Geometry: final body of the model. Coordinates: model frame, mm. Face numbers are marked on the shaded views. A direction names the side the tool comes from. Give positions to 0.01 mm unless a question says otherwise; leave off trailing zeros. Order: outer loops, then holes, each group sorted by start corner. A loop starts at its lowest first (then second) coordinate and runs counter-clockwise, first axis right, second up. Notation, with made-up numbers: (9, -37) - (44, -37) arc R13 cw to (44, -28) - close; hole circle Ø6 at (-29.5, 63.5). An arc over 180 degrees is marked (long way). Put each result on its own line as item: value. Start each with the question number.
1. Section D-D on y = 75. Return the cut outline in (x, z).
2. Mould query, pull axis Y, two halves, no side actions, for the marked faces 5, 6 and 7. Classes: pulls with the +Y half, pulls with the -Y half, needs draft (parallel to the pull), parting line crosses it, or undercut.
3. First-contact query: P1, Ø1.5, axis at x = -31, y = -5.5, coming from the -Z side; P2, Ø12, axis at y = 60, z = 4, coming from the -X side; P3, Ø7, axis at x = -39.5, z = -9.5, coming from the +Y side. Flat tips, straight axial feed; report the tip coordinate or a pass-through.
4. Section A-A on z = 0. Return the cut outline in (x, y), plus the area to 3 significant figures.
5. Ray query, line 1 along Y through (x, z) = (17, 0); line 2 along Y through (x, z) = (17, 20); line 3 along Z through (x, y) = (-16, -7.5). Return the intervals inside material, ascending. Write a range as from..to.
6. Set-up query: the marked faces 1, 2, 3 and 4. Return all of +Z, -Z, +X, -X, +Y, -Y with unobstructed straight access to the full face (end or side cutting, diameter ignored); none if empty.
7. Section C-C on x = 0. Return the cut outline in (y, z).
8. Section B-B on x = -21.5. Return the cut outline in (y, z), plus the area to 3 significant figures.
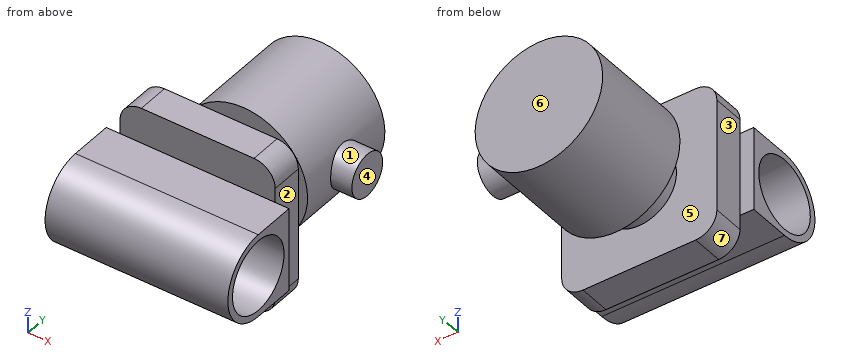
from build123d import *

# Parameters (mm, degrees)
SKETCH_1_R           = 19.75
SKETCH_1_R_2         = 16.75
EXTRUDE_1_DEPTH      = 43
EXTRUDE_1_2_DEPTH    = 15
SKETCH_4_R           = 17.5
EXTRUDE_2_DEPTH      = 15
SKETCH_5_R           = 30
EXTRUDE_3_DEPTH      = 50.25
EXTRUDE_START        = -86
EXTRUDE_4_DEPTH      = 86
EXTRUDE_5_REACH      = 137.171
EXTRUDE_5_END_RADIUS = 30
SKETCH_7_R           = 10


with BuildPart() as part:
    # Sketch 1 → Extrude 1 (new, symmetric)
    with BuildSketch(Plane(origin=(0, 0, 0), x_dir=(0, 0, -1), z_dir=(1, 0, 0))):
        Circle(SKETCH_1_R)
        Circle(SKETCH_1_R_2, mode=Mode.SUBTRACT)
    extrude(amount=EXTRUDE_1_DEPTH, both=True)



with BuildPart() as body_2:
    # Sketch 3 → Extrude 1 2 (new body)
    with BuildSketch(Plane(origin=(0, 20, 0), x_dir=(1, 0, 0), z_dir=(0, 1, 0))):
        with BuildLine():
            Line((-26.5, 36.5), (26.5, 36.5))
            ThreePointArc((26.5, 36.5), (33.571067812, 33.571067812), (36.5, 26.5))
            Line((36.5, 26.5), (36.5, -26.5))
            ThreePointArc((36.5, -26.5), (33.571067812, -33.571067812), (26.5, -36.5))
            Line((26.5, -36.5), (-26.5, -36.5))
            ThreePointArc((-26.5, -36.5), (-33.571067812, -33.571067812), (-36.5, -26.5))
            Line((-36.5, -26.5), (-36.5, 26.5))
            ThreePointArc((-36.5, 26.5), (-33.571067812, 33.571067812), (-26.5, 36.5))
        make_face()
    extrude(amount=EXTRUDE_1_2_DEPTH)

    # Sketch 4 → Extrude 2 (add)
    with BuildSketch(Plane(origin=(0, 35, 0), x_dir=(1, 0, 0), z_dir=(0, 1, 0))):
        with Locations(Location((0, 0, 0), (0, 0, 90))):
            Circle(SKETCH_4_R)
    extrude(amount=EXTRUDE_2_DEPTH)

    # Sketch 5 → Extrude 3 (add)
    with BuildSketch(Plane(origin=(0, 50, 0), x_dir=(1, 0, 0), z_dir=(0, 1, 0))):
        with Locations(Location((0, 0, 0), (0, 0, 270))):
            Circle(SKETCH_5_R)
    extrude(amount=EXTRUDE_3_DEPTH)


with BuildPart() as part_1:
    add(part.part)

    add(body_2.part)  # Extrude 4 merges body 2
    # Sketch 6 → Extrude 4 (add)
    with BuildSketch(Plane(origin=(43, 0, 0), x_dir=(0, 0, -1), z_dir=(1, 0, 0)).offset(EXTRUDE_START)):
        with BuildLine():
            Line((-19.75, 0), (-19.75, 20))
            Line((-19.75, 20), (19.75, 20))
            Line((19.75, 20), (19.75, 0))
            ThreePointArc((19.75, 0), (0, 19.75), (-19.75, 0))
        make_face()
    extrude(amount=EXTRUDE_4_DEPTH)

    # Extrude 5: up to this cylinder (the profile starts outside it)
    extrude_5_end = Plane(origin=(0, 75, 0), z_dir=(0, -1, 0)) * Cylinder(EXTRUDE_5_END_RADIUS, 335.342, mode=Mode.PRIVATE)
    # Sketch 7 → Extrude 5 (add, up to the surface)
    with BuildSketch(Plane(origin=(40, 0, 0), x_dir=(0, 0, -1), z_dir=(1, 0, 0)), mode=Mode.PRIVATE) as extrude_5_sk1:
        with Locations((0, 75)):
            Circle(SKETCH_7_R)
    extrude_5_tool1 = extrude(extrude_5_sk1.sketch, amount=-EXTRUDE_5_REACH, mode=Mode.PRIVATE) - extrude_5_end
    add(extrude_5_tool1.solids().sort_by_distance((40, 75, 0))[0])


solid = part_1.part
Resolved:
1. outline: (28.28, -10) - (40, -10) - (40, 10) - (28.28, 10) arc R30 ccw (long way) to start
2. face 5: undercut
2. face 6: pulls with the +Y half
2. face 7: needs draft
3. P1: z = -19.17
3. P2: x = -30
3. P3: y = 35
4. outline: (-43, -19.75) - (43, -19.75) - (43, -16.75) - (-43, -16.75) - close; (-43, 16.75) - (43, 16.75) - (43, 20) - (36.5, 20) - (36.5, 35) - (17.5, 35) - (17.5, 50) - (30, 50) - (30, 65) - (40, 65) - (40, 85) - (30, 85) - (30, 100.25) - (-30, 100.25) - (-30, 50) - (-17.5, 50) - (-17.5, 35) - (-36.5, 35) - (-36.5, 20) - (-43, 20) - close
4. area: 5,370 mm^2
5. line 1: -19.75..-16.75, 16.75..100.25
5. line 2: 20..35, 50..100.25
5. line 3: -18.27..-14.98, 14.98..18.27
6. face 1: +X
6. face 2: +Z, -Z, +X
6. face 3: +Z, -Z, -X, +Y
6. face 4: +Z, -Z, +X, +Y
7. outline: (0, -19.75) - (20, -19.75) - (20, -36.5) - (35, -36.5) - (35, -17.5) - (50, -17.5) - (50, -30) - (100.25, -30) - (100.25, 30) - (50, 30) - (50, 17.5) - (35, 17.5) - (35, 36.5) - (20, 36.5) - (20, 19.75) - (0, 19.75) arc R19.75 ccw to start; hole circle Ø33.5 at (0, 0)
8. outline: (0, -19.75) - (20, -19.75) - (20, -36.5) - (35, -36.5) - (35, 36.5) - (20, 36.5) - (20, 19.75) - (0, 19.75) arc R19.75 ccw to start; (50, -20.92) - (100.25, -20.92) - (100.25, 20.92) - (50, 20.92) - close; hole circle Ø33.5 at (0, 0)
8. area: 3,720 mm^2
